from build123d import *

# Parameters (mm, degrees)
SKETCH_1_R               = 42.5
EXTRUDE_1_DEPTH          = 80
SKETCH_2_R               = 57.5
EXTRUDE_2_DEPTH          = 10
SKETCH_3_OUTSIDE_W       = 154.176
SKETCH_3_OUTSIDE_H       = 154.176
SKETCH_3_OUTSIDE_W_2     = 85
SKETCH_3_OUTSIDE_H_2     = 85
CUT_EXTRUDE_1_DEPTH      = 122.295094707
SKETCH_4_R               = 35
CUT_EXTRUDE_2_DEPTH      = 8
PATTERN_CIRCULAR_1_COUNT = 4
SKETCH_7_R               = 32.5
CUT_EXTRUDE_3_DEPTH      = 102.668579217
CUT_EXTRUDE_4_DEPTH      = 109.22430411
CUT_EXTRUDE_4_DEPTH_BACK = 109.22430411
SKETCH_8_W               = 68
SKETCH_8_H               = 50
PATTERN_CIRCULAR_2_COUNT = 4


with BuildPart() as part:
    # 草图1 → 凸台-拉伸1 (new body)
    with BuildSketch(Plane(origin=(0, 0, 0), x_dir=(0, 0, -1), z_dir=(1, 0, 0))):
        Circle(SKETCH_1_R)
    extrude(amount=EXTRUDE_1_DEPTH)

    # 草图2 → 凸台-拉伸2 (add)
    with BuildSketch(Plane(origin=(80, 0, 0), x_dir=(0, 0, -1), z_dir=(1, 0, 0))):
        Circle(SKETCH_2_R)
    extrude(amount=EXTRUDE_2_DEPTH)

    # 草图3 outside → 切除-拉伸1 (cut, through all)
    with BuildSketch(Plane(origin=(90, 0, 0), x_dir=(0, 0, -1), z_dir=(1, 0, 0))):
        Rectangle(SKETCH_3_OUTSIDE_W, SKETCH_3_OUTSIDE_H)
        Rectangle(SKETCH_3_OUTSIDE_W_2, SKETCH_3_OUTSIDE_H_2, mode=Mode.SUBTRACT)
    extrude(amount=-CUT_EXTRUDE_1_DEPTH, mode=Mode.SUBTRACT)

    # 草图4 → 切除-拉伸2 (cut)
    with BuildSketch(Plane(origin=(90, 0, 0), x_dir=(0, 0, -1), z_dir=(1, 0, 0))):
        Circle(SKETCH_4_R)
    extrude(amount=-CUT_EXTRUDE_2_DEPTH, mode=Mode.SUBTRACT)

    # 草图6 → M6 螺纹孔1 (revolve, cut)
    with BuildSketch(Plane(origin=(90, 35.355339059, 35.355339059), x_dir=(0, 0, -1), z_dir=(0, 1, 0))):
        Polygon((0, 0), (0, 16.502151548), (2.5, 15), (2.5, 0), align=None)
    hole_wizard_m6_1 = revolve(axis=Axis((96.35, 35.355339059, 35.355339059), (-1, 0, 0)), mode=Mode.SUBTRACT)

    # 阵列(圆周)1: M6 螺纹孔1 ×4 about axis
    pattern_circular_1_axis = Axis((0, 0, 0), (1, 0, 0))
    for i in range(1, PATTERN_CIRCULAR_1_COUNT):
        add(hole_wizard_m6_1.rotate(pattern_circular_1_axis, i * 360 / PATTERN_CIRCULAR_1_COUNT), mode=Mode.SUBTRACT)

    # 草图7 → 切除-拉伸3 (cut, through all)
    with BuildSketch(Plane(origin=(82, 0, 0), x_dir=(0, 0, -1), z_dir=(1, 0, 0))):
        Circle(SKETCH_7_R)
    extrude(amount=-CUT_EXTRUDE_3_DEPTH, mode=Mode.SUBTRACT)

    # 草图8 → 切除-拉伸4 (cut, two sides: drawn at the far end of the back side and taken through both)
    with BuildSketch(Plane(origin=(0, 0, 0), x_dir=(1, 0, 0), z_dir=(0, 1, 0)).offset(-CUT_EXTRUDE_4_DEPTH_BACK)):
        with Locations((46, 0)):
            Rectangle(SKETCH_8_W, SKETCH_8_H)
    extrude(amount=CUT_EXTRUDE_4_DEPTH + CUT_EXTRUDE_4_DEPTH_BACK, mode=Mode.SUBTRACT)

    # 草图10 → M6 螺纹孔2 (revolve, cut)
    with BuildSketch(Plane(origin=(0, 26.162950904, -26.162950904), x_dir=(0, 0, 1), z_dir=(0, 1, 0))):
        Polygon((0, 0), (0, 16.502151548), (2.5, 15), (2.5, 0), align=None)
    hole_wizard_m6_2 = revolve(axis=Axis((-6.35, 26.162950904, -26.162950904), (1, 0, 0)), mode=Mode.SUBTRACT)

    # 阵列(圆周)2: M6 螺纹孔2 ×4 about axis
    pattern_circular_2_axis = Axis((0, 0, 0), (1, 0, 0))
    for i in range(1, PATTERN_CIRCULAR_2_COUNT):
        add(hole_wizard_m6_2.rotate(pattern_circular_2_axis, i * 360 / PATTERN_CIRCULAR_2_COUNT), mode=Mode.SUBTRACT)


solid = part.part
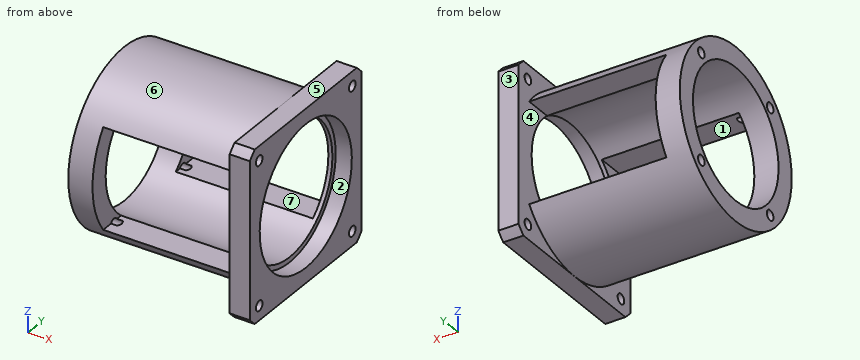
Geometry: final body of the model. Coordinates: model frame, mm. Face numbers are marked on the shaded views. A direction names the side the tool comes from. Round coordinates to 2 decimals unless told otherwise and drop trailing zeros. Write each loop counter-clockwise with the first axis right and the second up, starting at its lowest first coordinate (ties: lowest second). Pieces come first, ordered by that corner, then holes. Notation, with made-up numbers: M 67.25,7.25 L 95.25,7.25 A28 ccw 95.25,33.25 Z; hole C 68.5,42.5 d4. An arc over 180 degrees is marked long. Write item = value, one per line.
Item 1: Section query D-D on z = -9.5. Return loops of the section in (x, y), then the cut area to 3 significant figures.
Findings:
outline = M 0,-41.42 L 12,-41.42 L 12,-31.08 L 0,-31.08 Z; M 0,31.08 L 12,31.08 L 12,41.42 L 0,41.42 Z; M 80,-42.5 L 90,-42.5 L 90,-33.69 L 82,-33.69 L 82,-31.08 L 80,-31.08 Z; M 80,31.08 L 82,31.08 L 82,33.69 L 90,33.69 L 90,42.5 L 80,42.5 Z
area = 435 mm^2
Item 2: Section query C-C on y = 19.5. Return loops of the section in (x, z), then the cut area to 3 significant figures.
Findings:
outline = M 0,-37.76 L 80,-37.76 L 80,-42.5 L 90,-42.5 L 90,-29.06 L 82,-29.06 L 82,-26 L 0,-26 Z; M 0,26 L 82,26 L 82,29.06 L 90,29.06 L 90,42.5 L 80,42.5 L 80,37.76 L 0,37.76 Z
area = 2,160 mm^2
Item 3: Pull-direction query (Y, two-part tool) for the marked faces 1, 2 and 3; classes: pulls with the +Y half, pulls with the -Y half, needs draft (parallel to the pull), parting line crosses it, or undercut.
Findings:
face_1 = needs draft
face_2 = undercut
face_3 = pulls with the +Y half
Item 4: Section query A-A on z = 0. Return loops of the section in (x, y).
Findings:
outline = M 0,-42.5 L 12,-42.5 L 12,-32.5 L 0,-32.5 Z; M 0,32.5 L 12,32.5 L 12,42.5 L 0,42.5 Z; M 80,-42.5 L 90,-42.5 L 90,-35 L 82,-35 L 82,-32.5 L 80,-32.5 Z; M 80,32.5 L 82,32.5 L 82,35 L 90,35 L 90,42.5 L 80,42.5 Z
Item 5: Section query B-B on x = 22.5. Return loops of the section in (y, z), then the cut area to 3 significant figures.
Findings:
outline = M -34.37,-25 A42.5 ccw 34.37,-25 L 20.77,-25 A32.5 cw -20.77,-25 Z; M -34.37,25 L -20.77,25 A32.5 cw 20.77,25 L 34.37,25 A42.5 ccw Z
area = 1,260 mm^2
Item 6: Access query for the marked faces 4, 5, 6 and 7. Directions: +Z, -Z, +X, -X, +Y, -Y. A direction counts if a zero-diameter tool reaches every point of the face in a straight line with its end or side. Return the directions, or none.
Findings:
face_4 = +Y
face_5 = +Z, +X, -X, +Y, -Y
face_6 = -X
face_7 = +Y, -Y
Item 7: Pin query (flat end, axial travel): P1, Ø4.5, axis at y = 35.36, z = 35.36, coming from the +X side; P2, Ø12, axis at x = 37, y = 19.5, coming from the -Z side; P3, Ø15, axis at x = 47, y = -28.5, coming from the +Z side; P4, Ø4.5, axis at y = -26.16, z = -26.16, coming from the -X side. Return the tip coordinate at first contact, or that it passes through.
Findings:
P1 = through
P2 = -40.3
P3 = 36.95
P4 = 15.15
Item 8: Material intervals for line 1 along X through (y, z) = (30, -24.5); line 2 along X through (y, z) = (-31.5, 15); line 3 along X through (y, z) = (-10.5, -32.5), sorted ascending. Write a range as [from, to].
Findings:
line_1 = [0, 12], [80, 90]
line_2 = [0, 12], [80, 82]
line_3 = [0, 82]
